```python
from build123d import *

# Parameters (mm, degrees)
MAIN_BORE_PROFILE_28_18_R   = 14
MAIN_BORE_PROFILE_28_18_R_2 = 9
MAIN_BORE_TUBE_28X35_DEPTH  = 17.5
PIVOT_BOSS_PROFILE_15_9_R   = 7.5
PIVOT_BOSS_PROFILE_15_9_R_2 = 4.5
PIVOT_BOSS_15X19_DEPTH      = 9.5
SIDE_RIB_5MM_DEPTH          = 2.5
FRONT_RIB_5MM_DEPTH         = 2.5
FRONT_RIB_PAD_PROFILE_W     = 19
FRONT_RIB_PAD_PROFILE_H     = 5
FRONT_RIB_PAD_3MM_DEPTH     = 3
SIDE_RIB_PAD_PROFILE_W      = 5
SIDE_RIB_PAD_PROFILE_H      = 35
SIDE_RIB_PAD_3MM_DEPTH      = 3


with BuildPart() as part:
    # Main Bore Profile Ø28-Ø18 → Main Bore Tube Ø28x35 (new, symmetric)
    with BuildSketch(Plane.XY):
        Circle(MAIN_BORE_PROFILE_28_18_R)
        Circle(MAIN_BORE_PROFILE_28_18_R_2, mode=Mode.SUBTRACT)
    extrude(amount=MAIN_BORE_TUBE_28X35_DEPTH, both=True)



with BuildPart() as body_2:
    # Pivot Boss Profile Ø15-Ø9 → Pivot Boss Ø15x19 (new, symmetric)
    with BuildSketch(Plane(origin=(0, 0, 0), x_dir=(0, 0, -1), z_dir=(1, 0, 0))):
        with Locations((0, 26)):
            Circle(PIVOT_BOSS_PROFILE_15_9_R)
        with Locations((0, 26)):
            Circle(PIVOT_BOSS_PROFILE_15_9_R_2, mode=Mode.SUBTRACT)
    extrude(amount=PIVOT_BOSS_15X19_DEPTH, both=True)

    # Side Rib Profile → Side Rib 5mm (add, symmetric)
    with BuildSketch(Plane(origin=(0, 0, 0), x_dir=(0, 0, -1), z_dir=(1, 0, 0))):
        with BuildLine():
            Line((-17.5, 14), (-6.153967777, 30.287036342))
            ThreePointArc((-6.153967777, 30.287036342), (0, 18.5), (6.153967777, 30.287036342))
            Line((6.153967777, 30.287036342), (17.5, 14))
            Line((17.5, 14), (-17.5, 14))
        make_face()
    extrude(amount=SIDE_RIB_5MM_DEPTH, both=True)



with BuildPart() as body_3:
    # Front Rib Profile → Front Rib 5mm (new, symmetric)
    with BuildSketch(Plane.XY):
        with BuildLine():
            Line((-13.514557534, 3.654686672), (-9.5, 18.5))
            Line((-9.5, 18.5), (9.5, 18.5))
            Line((9.5, 18.5), (13.514557534, 3.654686672))
            ThreePointArc((13.514557534, 3.654686672), (0, 14), (-13.514557534, 3.654686672))
        make_face()
    extrude(amount=FRONT_RIB_5MM_DEPTH, both=True)


with BuildPart() as body_2_1:
    add(body_2.part)

    add(body_3.part)  # Front Rib Pad 3mm merges body 3
    # Front Rib Pad Profile → Front Rib Pad 3mm (add)
    with BuildSketch(Plane(origin=(0, 18.5, 0), x_dir=(1, 0, 0), z_dir=(0, 1, 0))):
        Rectangle(FRONT_RIB_PAD_PROFILE_W, FRONT_RIB_PAD_PROFILE_H)
    extrude(amount=FRONT_RIB_PAD_3MM_DEPTH)


with BuildPart() as part_1:
    add(part.part)

    add(body_2_1.part)  # Side Rib Pad 3mm merges body 2
    # Side Rib Pad Profile → Side Rib Pad 3mm (add)
    with BuildSketch(Plane.XZ.offset(-14)):
        Rectangle(SIDE_RIB_PAD_PROFILE_W, SIDE_RIB_PAD_PROFILE_H)
    extrude(amount=SIDE_RIB_PAD_3MM_DEPTH)


solid = part_1.part
```
Input: part model. Units: mm. Frame: model coordinates. A direction names the side the tool comes from. Round coordinates to 2 decimals unless told otherwise and drop trailing zeros. Order: outer loops, then holes, each group sorted by start corner. A loop starts at its lowest first (then second) coordinate and runs counter-clockwise, first axis right, second up. Notation, with made-up numbers: (32.5, 11.25) - (45.5, 11.25) arc R21 cw to (45.5, 41.25) - close; hole circle Ø4 at (0, 87). An arc over 180 degrees is marked (long way). One line per question, with ' | ' between items. Start each with the question number.
1) Cut plane C-C, the plane y = 0. Return the cut outline in (x, z), then the cut area to 3 significant figures.
2) Ray query, probe 1 along Z at (x, y) = (9.75, 15.5); probe 2 along Y at (x, z) = (0, -5.5). Return the intervals inside material, ascending.
3) Set-up query: faces 1 (the flat face through (-9.5, 26, -5)), 2 (the flat face through (2.5, 18, -8)), 3 (the cylindrical face through (0.133, 33.494, -0.294)). Return all of +Z, -Z, +X, -X, +Y, -Y with unobstructed straight access to the full face (end or side cutting, diameter ignored); none if empty.
4) Contact query for flat-ended pins moving along their axis: P1, Ø4, axis at y = 8.5, z = -10.5, coming from the +X side; P2, Ø7.5, axis at y = 25.5, z = -12.5, coming from the +X side; P3, Ø4, axis at y = -3.5, z = -13.5, coming from the +X side; P4, Ø5.5, axis at y = 26, z = 0, coming from the +X side. Output: stop coordinate, or through.
5) Cut plane B-B, the plane z = 0. Return the cut outline in (x, y), then the cut area to 3 significant figures.
6) Pull-direction query (X, two-part tool) for faces 4 (the flat face through (-2.5, 18, -8)), 5 (the cylindrical face through (-1.172, 8.923, -0.245)), 6 (the flat face through (-8, 14, 2.5)); classes: +X half, -X half, draft (parallel to the pull), parting line (faces both ways), or undercut.
7) Cut plane A-A, the plane x = 0. Return the cut outline in (y, z), then the cut area to 3 significant figures.
8) Cut plane D-D, the plane x = 4.5. Return the cut outline in (y, z), then the cut area to 3 significant figures.
Worked out:
1) outline: (-14, -17.5) - (-9, -17.5) - (-9, 17.5) - (-14, 17.5) - close; (9, -17.5) - (14, -17.5) - (14, 17.5) - (9, 17.5) - close | area: 350 mm^2
2) probe 1: z = -2.5 to 2.5 | probe 2: y = -14 to -9, 9 to 31.1
3) face 1: +Z, -Z, -X, +Y | face 2: -Z, +X | face 3: none
4) P1: stops at x = 12.4 | P2: stops at x = 2.5 | P3: stops at x = 13.92 | P4: passes through
5) outline: (-13.51, 3.65) arc R14 ccw (long way) to (13.51, 3.65) - (9.5, 18.5) - (9.5, 21.5) - (-9.5, 21.5) - (-9.5, 18.5) - close; (-9.5, 30.5) - (9.5, 30.5) - (9.5, 33.5) - (-9.5, 33.5) - close; hole circle Ø18 at (0, 0) | area: 610 mm^2
6) face 4: -X half | face 5: undercut | face 6: draft
7) outline: (-14, -17.5) - (-9, -17.5) - (-9, 17.5) - (-14, 17.5) - close; (9, -17.5) - (14, -17.5) - (30.29, -6.15) arc R7.5 ccw to (30.29, 6.15) - (14, 17.5) - (9, 17.5) - close; hole circle Ø9 at (26, 0) | area: 699 mm^2
8) outline: (-13.26, -17.5) - (-7.79, -17.5) - (-7.79, 17.5) - (-13.26, 17.5) - close; (7.79, -17.5) - (13.26, -17.5) - (13.26, -2.5) - (18.93, -2.5) arc R7.5 ccw (long way) to (18.93, 2.5) - (13.26, 2.5) - (13.26, 17.5) - (7.79, 17.5) - close; hole circle Ø9 at (26, 0) | area: 522 mm^2
